```python
from build123d import *

# Parameters (mm, degrees)
SKETCH_1_W          = 120
SKETCH_1_H          = 45
EXTRUDE_1_DEPTH     = 15
SKETCH_2_W          = 170
SKETCH_2_H          = 52
EXTRUDE_2_DEPTH     = 4
SKETCH_3_R          = 5.5
CUT_EXTRUDE_1_DEPTH = 97.669540187


with BuildPart() as part:
    # 草图1 → 凸台-拉伸1 (new, symmetric)
    with BuildSketch(Plane.XY):
        Rectangle(SKETCH_1_W, SKETCH_1_H)
    extrude(amount=EXTRUDE_1_DEPTH, both=True)

    # 草图2 → 凸台-拉伸2 (add)
    with BuildSketch(Plane.XY.offset(15)):
        Rectangle(SKETCH_2_W, SKETCH_2_H)
    extrude_2 = extrude(amount=EXTRUDE_2_DEPTH)

    # 镜向1: 凸台-拉伸2 across plane
    add(extrude_2.mirror(Plane.XY))

    # 草图3 → 切除-拉伸1 (cut, through all)
    with BuildSketch(Plane.XY.offset(19)):
        with Locations((-75, 0)):
            Circle(SKETCH_3_R)
        with Locations(Location((75, 0, 0), (0, 0, 180))):
            Circle(SKETCH_3_R)
    extrude(amount=-CUT_EXTRUDE_1_DEPTH, mode=Mode.SUBTRACT)


solid = part.part
```
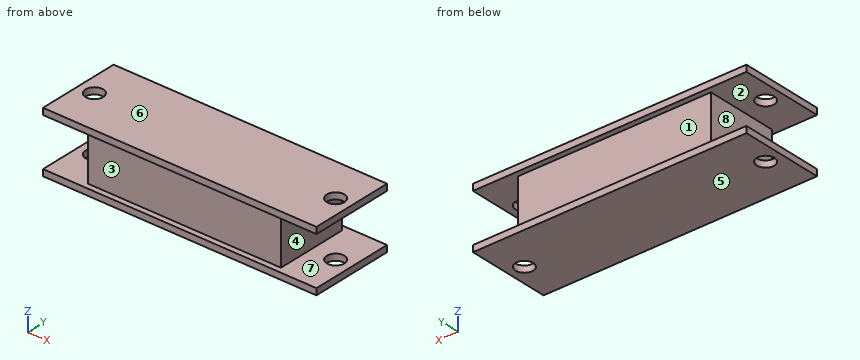
Geometry check sheet. Reference: the model listing, model coordinates, mm. Face numbers are marked on the shaded views. A direction names the side the tool comes from. Give positions to 0.01 mm unless a question says otherwise; leave off trailing zeros. Write each loop counter-clockwise with the first axis right and the second up, starting at its lowest first coordinate (ties: lowest second). Pieces come first, ordered by that corner, then holes.
1) Gauge pin test, flat ends, axial feed: pin 1 (8 mm diameter, centred on y = -20, z = 9.5, fed in from +X); pin 2 (10 mm diameter, centred on x = 18, z = -2, fed in from +Y); pin 3 (10 mm diameter, centred on y = -17.5, z = -6, fed in from -X). Record the tip position at first contact, or that the pin passes through.
2) Section check D-D, the plane y = 19. Record the boundary of the cut face in (x, z).
3) Section check B-B, the plane x = 64. Record the boundary of the cut face in (y, z).
4) Material ranges on L1, parallel to Y at x = -75, z = 16; L2, parallel to X at y = 8.5, z = -3; L3, parallel to Y at x = -12.5, z = -13.5, recorded low to high.
5) Release check for a two-part mould opening along Z. For the marked faces 5, 6, 7 and 8 record: pulls with the +Z half, pulls with the -Z half, needs draft (parallel to the pull), parting line crosses it, or undercut.
6) Access from +Z, -Z, +X, -X, +Y, -Y to the whole of each face (thin tool, end or side, straight path). Record for the marked faces 1, 2, 3 and 4.
7) Section check A-A, the plane y = 0. Record the boundary of the cut face in (x, z).
8) Section check C-C, the plane x = -38.5. Record the boundary of the cut face in (y, z).
Computed:
1. pin 1: stops at x = 60
1. pin 2: stops at y = 22.5
1. pin 3: stops at x = -60
2. outline: (-85, -19) - (85, -19) - (85, -15) - (60, -15) - (60, 15) - (85, 15) - (85, 19) - (-85, 19) - (-85, 15) - (-60, 15) - (-60, -15) - (-85, -15) - close
3. outline: (-26, -19) - (26, -19) - (26, -15) - (-26, -15) - close; (-26, 15) - (26, 15) - (26, 19) - (-26, 19) - close
4. L1: y = -26 to -5.5, 5.5 to 26
4. L2: x = -60 to 60
4. L3: y = -22.5 to 22.5
5. face 5: pulls with the -Z half
5. face 6: pulls with the +Z half
5. face 7: undercut
5. face 8: undercut
6. face 1: +X, -X, +Y
6. face 2: none
6. face 3: +X, -X, -Y
6. face 4: +X, +Y, -Y
7. outline: (-85, -19) - (-80.5, -19) - (-80.5, -15) - (-85, -15) - close; (-85, 15) - (-80.5, 15) - (-80.5, 19) - (-85, 19) - close; (-69.5, -19) - (69.5, -19) - (69.5, -15) - (60, -15) - (60, 15) - (69.5, 15) - (69.5, 19) - (-69.5, 19) - (-69.5, 15) - (-60, 15) - (-60, -15) - (-69.5, -15) - close; (80.5, -19) - (85, -19) - (85, -15) - (80.5, -15) - close; (80.5, 15) - (85, 15) - (85, 19) - (80.5, 19) - close
8. outline: (-26, -19) - (26, -19) - (26, -15) - (22.5, -15) - (22.5, 15) - (26, 15) - (26, 19) - (-26, 19) - (-26, 15) - (-22.5, 15) - (-22.5, -15) - (-26, -15) - close
